Build history of the part. All positions in model axes, mm. Give positions to 0.01 mm unless a question says otherwise; leave off trailing zeros. Write each loop counter-clockwise with the first axis right and the second up, starting at its lowest first coordinate (ties: lowest second). Pieces come first, ordered by that corner, then holes. Notation, with made-up numbers: (-10.5, 86.25) -> (1.5, 86.25) arc R26 cw to (1.5, 125.25) -> close; hole circle Ø8 at (41, 2). An arc over 180 degrees is marked (long way). One line per question, with ' | ' between items. Start each with the question number.
(1) Band-saw the part on A-A, the plane z = 4. Give the cut face in (x, y), and give its area (3 significant figures).
(2) Pin check, flat tip, straight feed: P1, Ø3, axis at y = 2, z = 4, coming from the -X side. Stop position of the tip, or through.
(3) Drill centre lines: probe 1 along Y at (x, z) = (5.5, 2.2); probe 2 along X at (y, z) = (-2.55, 0.6); probe 3 along X at (y, z) = (-1.75, 1.7). Where is each one in solid material? Low to high. Write a range as from..to.
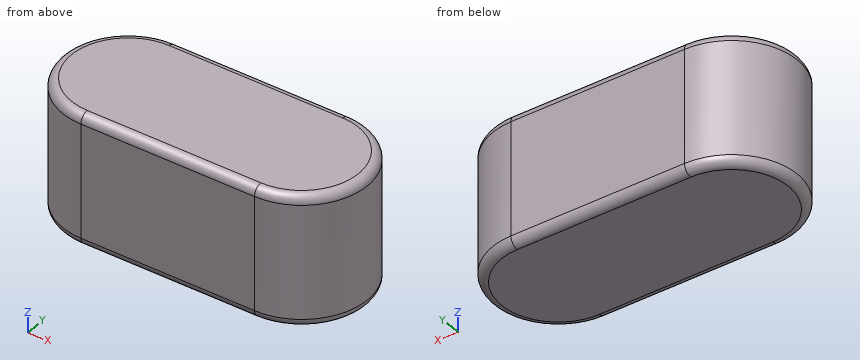
from build123d import *

# Parameters (mm, degrees)
EXTRUDE_523_DEPTH = 6
FILLET_1_R        = 0.4


with BuildPart() as part:
    # 草图1 → Extrude 523 (new body)
    with BuildSketch(Plane.XY):
        with BuildLine():
            Line((-4, 3), (4, 3))
            ThreePointArc((4, 3), (7, 0), (4, -3))
            Line((4, -3), (-4, -3))
            ThreePointArc((-4, -3), (-7, 0), (-4, 3))
        make_face()
    extrude(amount=EXTRUDE_523_DEPTH)

    # 圆角1
    fillet_1_edges = [part.edges().sort_by_distance(p)[0] for p in [
        (7, 0, 6),
        (0, 3, 6),
        (-7, 0, 6),
        (0, 3, 0),
        (7, 0, 0),
        (0, -3, 0),
        (-7, 0, 0),
        (0, -3, 6),
    ]]
    fillet(fillet_1_edges, radius=FILLET_1_R)


solid = part.part
Results:
1) outline: (-4, -3) -> (4, -3) arc R3 ccw to (4, 3) -> (-4, 3) arc R3 ccw to start | area: 76.3 mm²
2) P1: stops at x = -6.96
3) probe 1: y = -2.6..2.6 | probe 2: x = -5.58..5.58 | probe 3: x = -6.44..6.44
